Verification items for the finished model (mm, model axes). Round coordinates to 2 decimals unless told otherwise and drop trailing zeros. Write each loop counter-clockwise with the first axis right and the second up, starting at its lowest first coordinate (ties: lowest second). Pieces come first, ordered by that corner, then holes. Notation, with made-up numbers: M -24.75,21.5 L -13.75,21.5 A16 cw -13.75,40.5 Z; hole C 67,17 d11. An arc over 180 degrees is marked long. Answer in a Markdown table with one row per item. Add a question column.
1. Sectioned sample at C-C on z = 0.6. Record the cut outline in (x, y), plus the area to 3 significant figures.
2. Sectioned sample at B-B on y = 660. Record the cut outline in (x, z), plus the area to 3 significant figures.
3. Go/stop test with a flat-tipped pin: pin 1 Ø0.9 at (y, z) = (489.5, 1) entering from -X. Record where the tip stops, or that it passes through.
4. Sectioned sample at D-D on x = 185.5. Record the cut outline in (y, z).
5. Material ranges on probe 1 along Y at (x, z) = (90, 1.7); probe 2 along Y at (x, z) = (138, 1.05); probe 3 along Y at (x, z) = (466, 0.35), recorded low to high.
6. Sectioned sample at A-A on x = 90. Record the cut outline in (y, z).
```python
from build123d import *

# Parameters (mm, degrees)
BOSS_EXTRUDE1_DEPTH = 3
SKETCH2_R           = 60
SKETCH2_W           = 120
SKETCH2_H           = 120
CUT_EXTRUDE1_DEPTH  = 10


with BuildPart() as part:
    # Sketch1 → Boss-Extrude1 (new body)
    with BuildSketch(Plane.XY):
        Polygon((0, 0), (530, 0), (530, 1165), (0, 1165), (0, 550), (300, 550), (300, 340), (0, 340), align=None)
    extrude(amount=BOSS_EXTRUDE1_DEPTH)

    # Sketch2 → Cut-Extrude1 (cut)
    with BuildSketch(Plane(origin=(0, 0, 0), x_dir=(-1, 0, 0), z_dir=(0, 0, -1))):
        with Locations((-90, 660)):
            Circle(SKETCH2_R)
        with Locations((-490, 660)):
            Rectangle(SKETCH2_W, SKETCH2_H)
    extrude(amount=-CUT_EXTRUDE1_DEPTH, mode=Mode.SUBTRACT)


solid = part.part
```
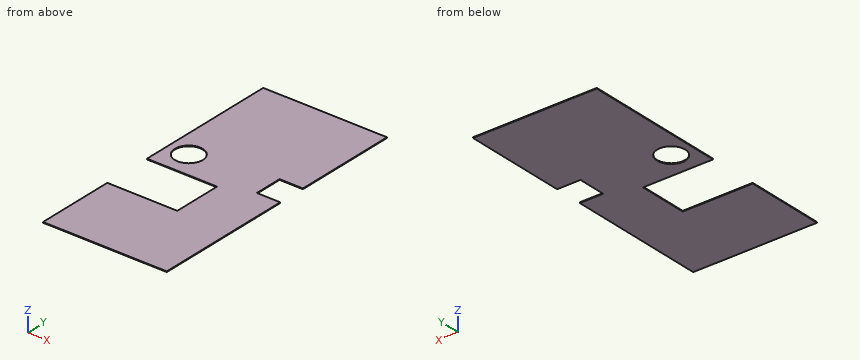
Geometry check:
| question | item | result |
|---|---|---|
| 1 | outline | M 0,0 L 530,0 L 530,600 L 430,600 L 430,720 L 530,720 L 530,1165 L 0,1165 L 0,550 L 300,550 L 300,340 L 0,340 Z; hole C 90,660 d120 |
| 1 | area | 531,000 mm2 |
| 2 | outline | M 0,0 L 30,0 L 30,3 L 0,3 Z; M 150,0 L 430,0 L 430,3 L 150,3 Z |
| 2 | area | 930 mm2 |
| 3 | pin 1 | stops at x = 300 |
| 4 | outline | M 0,0 L 340,0 L 340,3 L 0,3 Z; M 550,0 L 1165,0 L 1165,3 L 550,3 Z |
| 5 | probe 1 | y = 0 to 340, 550 to 600, 720 to 1165 |
| 5 | probe 2 | y = 0 to 340, 550 to 624, 696 to 1165 |
| 5 | probe 3 | y = 0 to 600, 720 to 1165 |
| 6 | outline | M 0,0 L 340,0 L 340,3 L 0,3 Z; M 550,0 L 600,0 L 600,3 L 550,3 Z; M 720,0 L 1165,0 L 1165,3 L 720,3 Z |
